```python
from build123d import *

# Parameters (mm, degrees)
SKETCH1_R           = 70
SKETCH1_R_2         = 50
BOSS_EXTRUDE1_DEPTH = 0.5
SKETCH2_R           = 4.5
CUT_EXTRUDE1_DEPTH  = 99.996212049
CIRPATTERN1_COUNT   = 6


with BuildPart() as part:
    # Sketch1 → Boss-Extrude1 (new body)
    with BuildSketch(Plane.XY):
        Circle(SKETCH1_R)
        Circle(SKETCH1_R_2, mode=Mode.SUBTRACT)
    extrude(amount=BOSS_EXTRUDE1_DEPTH)

    # Sketch2 → Cut-Extrude1 (cut, through all)
    with BuildSketch(Plane.XY.offset(0.5)):
        with Locations((0, 60)):
            Circle(SKETCH2_R)
    cut_extrude1 = extrude(amount=-CUT_EXTRUDE1_DEPTH, mode=Mode.SUBTRACT)

    # CirPattern1: Cut-Extrude1 ×6 about axis
    cirpattern1_axis = Axis((0, 0, 0), (0, 0, 1))
    for i in range(1, CIRPATTERN1_COUNT):
        add(cut_extrude1.rotate(cirpattern1_axis, i * 360 / CIRPATTERN1_COUNT), mode=Mode.SUBTRACT)


solid = part.part
```
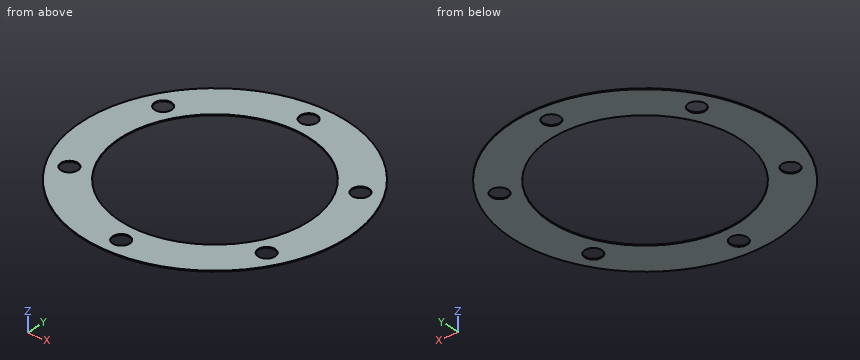
Geometry: final body of the model. Coordinates: model frame, mm. Coordinates: 2 decimals unless noted, no trailing zeros. Order: outer loops, then holes, each group sorted by start corner. A loop starts at its lowest first (then second) coordinate and runs counter-clockwise, first axis right, second up.
Item 1: Contact query for a flat-ended pin moving along its axis: P1, Ø11.5, axis at x = -51.96, y = -30, coming from the -Z side. Output: stop coordinate, or through.
Answer:
P1: stops at z = 0
Item 2: Section query A-A (x = 0). Output: boundary loops of the cut face in (y, z).
Answer:
outline: (-70, 0) - (-64.5, 0) - (-64.5, 0.5) - (-70, 0.5) - close; (-55.5, 0) - (-50, 0) - (-50, 0.5) - (-55.5, 0.5) - close; (50, 0) - (55.5, 0) - (55.5, 0.5) - (50, 0.5) - close; (64.5, 0) - (70, 0) - (70, 0.5) - (64.5, 0.5) - close
Item 3: Material intervals for line 1 along Y through (x, z) = (0, 0.2); line 2 along Y through (x, z) = (2, 0.4); line 3 along Y through (x, z) = (-17.5, 0.3), sorted ascending.
Answer:
line 1: y = -70 to -64.5, -55.5 to -50, 50 to 55.5, 64.5 to 70
line 2: y = -69.97 to -64.03, -55.97 to -49.96, 49.96 to 55.97, 64.03 to 69.97
line 3: y = -67.78 to -46.84, 46.84 to 67.78
Item 4: Section query C-C (x = 23.5). Output: boundary loops of the cut face in (y, z).
Answer:
outline: (-65.94, 0) - (-44.13, 0) - (-44.13, 0.5) - (-65.94, 0.5) - close; (44.13, 0) - (65.94, 0) - (65.94, 0.5) - (44.13, 0.5) - close
Item 5: Section query D-D (y = -8.5). Output: boundary loops of the cut face in (x, z).
Answer:
outline: (-69.48, 0) - (-49.27, 0) - (-49.27, 0.5) - (-69.48, 0.5) - close; (49.27, 0) - (69.48, 0) - (69.48, 0.5) - (49.27, 0.5) - close
Item 6: Section query B-B (y = -30). Output: boundary loops of the cut face in (x, z), then the cut area to 3 significant figures.
Answer:
outline: (-63.25, 0) - (-56.46, 0) - (-56.46, 0.5) - (-63.25, 0.5) - close; (-47.46, 0) - (-40, 0) - (-40, 0.5) - (-47.46, 0.5) - close; (40, 0) - (47.46, 0) - (47.46, 0.5) - (40, 0.5) - close; (56.46, 0) - (63.25, 0) - (63.25, 0.5) - (56.46, 0.5) - close
area: 14.2 mm2
